```python
from build123d import *

# Parameters (mm, degrees)
SKETCH_1_R      = 3
SKETCH_1_R_2    = 1.5
EXTRUDE_1_DEPTH = 60
EXTRUDE_START   = -3
SKETCH_2_R      = 5
SKETCH_2_R_2    = 1.5
EXTRUDE_2_DEPTH = 3
FILLET_1_R      = 0.5
CHAMFER_1_SIZE  = 0.5


with BuildPart() as part:
    # 草图1 → 凸台-拉伸1 (new body)
    with BuildSketch(Plane(origin=(0, 0, 0), x_dir=(1, 0, 0), z_dir=(0, 1, 0))):
        with Locations(Location((0, 0, 0), (0, 0, 270))):
            Circle(SKETCH_1_R)
        with Locations(Location((0, 0, 0), (0, 0, 270))):
            Circle(SKETCH_1_R_2, mode=Mode.SUBTRACT)
    extrude(amount=EXTRUDE_1_DEPTH)

    # 草图2 → 凸台-拉伸2 (add)
    with BuildSketch(Plane(origin=(0, 60, 0), x_dir=(1, 0, 0), z_dir=(0, 1, 0)).offset(EXTRUDE_START)):
        with Locations(Location((0, 0, 0), (0, 0, 270))):
            Circle(SKETCH_2_R)
        with Locations(Location((0, 0, 0), (0, 0, 270))):
            Circle(SKETCH_2_R_2, mode=Mode.SUBTRACT)
    extrude(amount=EXTRUDE_2_DEPTH)

    # 圆角1
    fillet_1_edges = [part.edges().sort_by_distance(p)[0] for p in [
        (0, 0, -1.5),
        (0, 60, -1.5),
    ]]
    fillet(fillet_1_edges, radius=FILLET_1_R)

    # 倒角1
    chamfer_1_edges = [part.edges().sort_by_distance(p)[0] for p in [
        (0, 60, -5),
        (0, 57, -5),
        (0, 0, -3),
    ]]
    chamfer(chamfer_1_edges, length=CHAMFER_1_SIZE)


solid = part.part
```
Input: part model. Units: mm. Frame: model coordinates. A direction names the side the tool comes from. Give positions to 0.01 mm unless a question says otherwise; leave off trailing zeros. Order: outer loops, then holes, each group sorted by start corner. A loop starts at its lowest first (then second) coordinate and runs counter-clockwise, first axis right, second up. Notation, with made-up numbers: (19, 33) -> (45, 33) arc R22 ccw to (45, 68) -> close; hole circle Ø5 at (70, 67). An arc over 180 degrees is marked (long way). Write each question's results on one line, items separated by ' | '. Start each with the question number.
Item 1: Set-up query: faces 1 (the flat face through (-2, 60, 1)), 2 (the flat face through (-3, 57, 1)). Return all of +Z, -Z, +X, -X, +Y, -Y with unobstructed straight access to the full face (end or side cutting, diameter ignored); none if empty.
Item 2: Cut plane B-B on x = 0. Return the cut outline in (y, z).
Item 3: Mould query, pull axis Z, two halves, no side actions, for faces 3 (the flat face through (2, 0, -1)), 4 (the cylindrical face through (0.45, 29.59, 1.43)), 5 (the cylindrical face through (-4.88, 58.49, -1.08)). Classes: pulls with the +Z half, pulls with the -Z half, needs draft (parallel to the pull), parting line crosses it, or undercut.
Item 4: Cut plane A-A on z = 0. Return the cut outline in (x, y).
Item 5: Cut plane C-C on y = 31. Return the cut outline in (x, z), then the cut area to 3 significant figures.
Item 6: Line query: line 1 (X direction, y = 23, z = 0); line 2 (Y direction, x = 2.25, z = -3.25); line 3 (Z direction, x = 0.25, y = 28). Output: solid intervals per line, ascending.
Item 7: Contact query for flat-ended pins moving along their axis: P1, Ø1.5, axis at x = 0, y = 27.5, coming from the +Z side; P2, Ø1.5, axis at x = -2.5, y = 10.5, coming from the -Z side; P3, Ø3, axis at x = -0.5, z = 1, coming from the +Y side; P4, Ø5, axis at x = 3, y = 22.5, coming from the -Z side. Output: stop coordinate, or through.
Established:
1) face 1: +Z, -Z, +X, -X, +Y | face 2: -Y
2) outline: (0, -2.5) -> (0.5, -3) -> (57, -3) -> (57, -4.5) -> (57.5, -5) -> (59.5, -5) -> (60, -4.5) -> (60, -2) arc R0.5 ccw to (59.5, -1.5) -> (0.5, -1.5) arc R0.5 ccw to (0, -2) -> close; (0, 2) arc R0.5 ccw to (0.5, 1.5) -> (59.5, 1.5) arc R0.5 ccw to (60, 2) -> (60, 4.5) -> (59.5, 5) -> (57.5, 5) -> (57, 4.5) -> (57, 3) -> (0.5, 3) -> (0, 2.5) -> close
3) face 3: needs draft | face 4: undercut | face 5: parting line crosses it
4) outline: (-5, 57.5) -> (-4.5, 57) -> (-3, 57) -> (-3, 0.5) -> (-2.5, 0) -> (-2, 0) arc R0.5 ccw to (-1.5, 0.5) -> (-1.5, 59.5) arc R0.5 ccw to (-2, 60) -> (-4.5, 60) -> (-5, 59.5) -> close; (1.5, 0.5) arc R0.5 ccw to (2, 0) -> (2.5, 0) -> (3, 0.5) -> (3, 57) -> (4.5, 57) -> (5, 57.5) -> (5, 59.5) -> (4.5, 60) -> (2, 60) arc R0.5 ccw to (1.5, 59.5) -> close
5) outline: circle Ø6 at (0, 0); hole circle Ø3 at (0, 0) | area: 21.2 mm^2
6) line 1: -3 to -1.5, 1.5 to 3 | line 2: 57 to 60 | line 3: -2.99 to -1.48, 1.48 to 2.99
7) P1: z = 3 | P2: z = -2.44 | P3: y = 60 | P4: z = -2.96
